The figure shows three views and two pictorial views of one solid part (mm, origin at its lowest corner). Answer the questions. A direction names the side the tool comes from. Coordinates: 2 decimals unless noted, no trailing zeros. Write each loop counter-clockwise with the first axis right and the second up, starting at its lowest first coordinate (ties: lowest second). Pieces come first, ordered by that corner, then holes. Notation, with made-up numbers: M 85.5,49.5 L 112.5,49.5 A30 ccw 112.5,72.5 Z; hole C -22.75,27 d9. An arc over 180 degrees is marked long. Use a Markdown table: item, result. Add a question column.
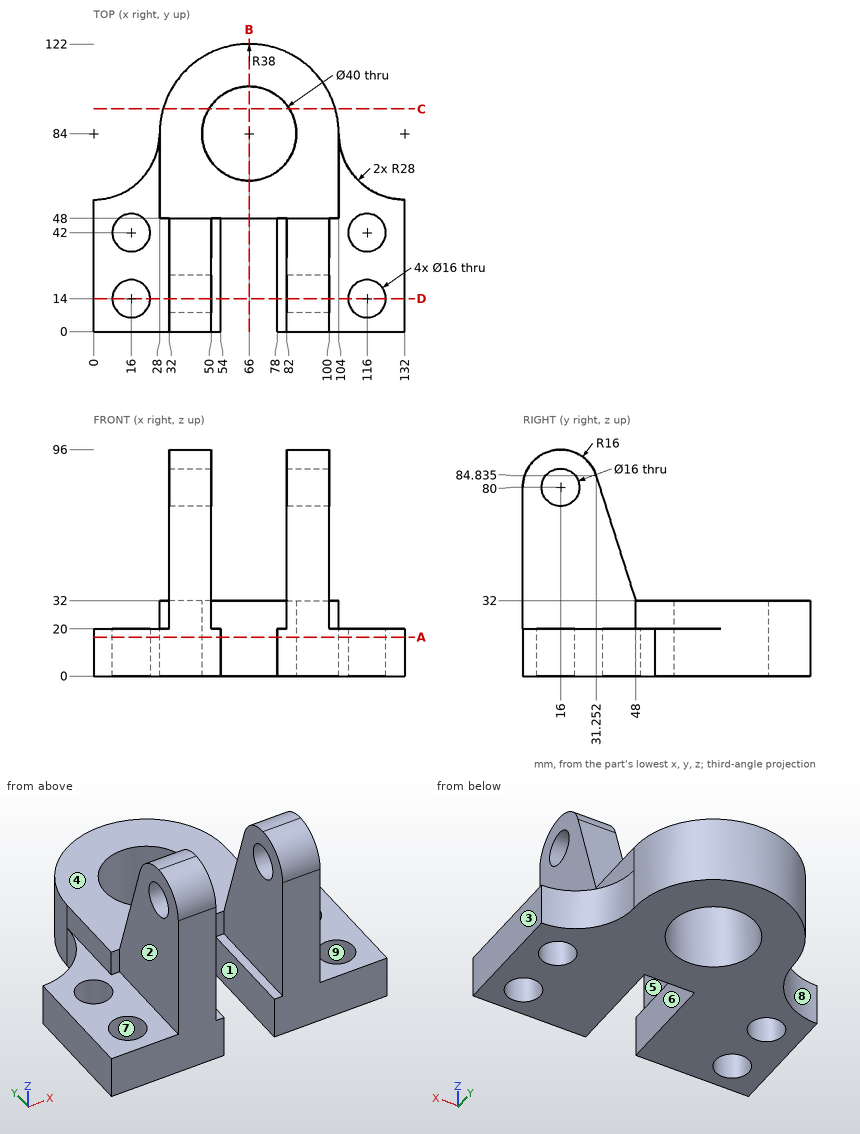
Item 1: Determine the mould class of the marked faces 6, 7, 8 and 9 for opening direction Y: pulls with the +Y half, pulls with the -Y half, needs draft (parallel to the pull), parting line crosses it, or undercut.
Item 2: Consider probe 1 along Y at (x, z) = (66, 23); probe 2 along X at (y, z) = (34.5, 54); probe 3 along Z at (x, y) = (48.5, 97.5). Determine where each line is inside the solid, lowest interval first.
Item 3: For the marked faces 1, 2, 3, 4 and 5, determine the directions among +Z, -Z, +X, -X, +Y, -Y from which every point of the face is accessible in a straight line to the end or side of a thin tool.
Item 4: Find section B-B on x = 66. Give the vertices of the cut face in (y, z), then the cut area to 3 significant figures.
Item 5: Each of these flat-tipped pins is pushed along its axis until it touches: pin 1 (1.2 mm diameter, centred on x = 30.5, z = 23.5, fed in from -Y); pin 2 (14.5 mm diameter, centred on y = 15, z = 39.5, fed in from +X); pin 3 (12 mm diameter, centred on x = 112, y = 80.5, fed in from +Z); pin 4 (3 mm diameter, centred on y = 24.5, z = 40, fed in from -X). Where does it stop, or does it pass through?
Item 6: Find section C-C on y = 94.5. Give the vertices of the cut face in (x, z).
Item 7: Find section D-D on y = 14. Count the separate pieces of the cut face and the enclosed holes in it, then the cut area to 3 significant figures.
Item 8: Find section A-A on z = 16.5. Give the vertices of the cut face in (x, y).
Geometry says:
| question | item | result |
|---|---|---|
| 1 | face 6 | needs draft |
| 1 | face 7 | undercut |
| 1 | face 8 | pulls with the +Y half |
| 1 | face 9 | undercut |
| 2 | probe 1 | y = 48 to 64, 104 to 122 |
| 2 | probe 2 | x = 32 to 50, 82 to 100 |
| 2 | probe 3 | z = 0 to 32 |
| 3 | face 1 | +Z, -Z, -Y |
| 3 | face 2 | +Z, -X, -Y |
| 3 | face 3 | +Z, -Z, +X, +Y, -Y |
| 3 | face 4 | +Z, +X, -X, +Y |
| 3 | face 5 | +Z, -Y |
| 4 | outline | M 48,0 L 64,0 L 64,32 L 48,32 Z; M 104,0 L 122,0 L 122,32 L 104,32 Z |
| 4 | area | 1,090 mm2 |
| 5 | pin 1 | stops at y = 48 |
| 5 | pin 2 | stops at x = 100 |
| 5 | pin 3 | passes through |
| 5 | pin 4 | stops at x = 32 |
| 6 | outline | M 29.48,0 L 48.98,0 L 48.98,32 L 29.48,32 Z; M 83.02,0 L 102.52,0 L 102.52,32 L 83.02,32 Z |
| 7 | separate pieces | 6 |
| 7 | enclosed holes | 0 |
| 7 | area | 3,690 mm2 |
| 8 | outline | M 0,0 L 54,0 L 54,48 L 78,48 L 78,0 L 132,0 L 132,56 A28 cw 104,84 A38 ccw 28,84 A28 cw 0,56 Z; hole C 16,14 d16; hole C 16,42 d16; hole C 66,84 d40; hole C 116,14 d16; hole C 116,42 d16 |
